Input: part model. Units: mm. Frame: model coordinates. A direction names the side the tool comes from. Round coordinates to 2 decimals unless told otherwise and drop trailing zeros. Order: outer loops, then holes, each group sorted by start corner. A loop starts at its lowest first (then second) coordinate and runs counter-clockwise, first axis right, second up. Notation, with made-up numbers: (4.5, -4.75) -> (48.5, -4.75) arc R21 cw to (48.5, 10.25) -> close; hole circle Ø1 at (23.5, 1.5). An arc over 180 degrees is marked (long way). Use a Markdown table: item, result.
from build123d import *

# Parameters (mm, degrees)
SKETCH1_R           = 35
SKETCH1_R_2         = 27.75
BOSS_EXTRUDE1_DEPTH = 6.5
CUT_EXTRUDE1_DEPTH  = 50.922439844
CHAMFER1_SIZE       = 2
CHAMFER2_SIZE       = 0.5


with BuildPart() as part:
    # Sketch1 → Boss-Extrude1 (new body)
    with BuildSketch(Plane.XY):
        with Locations(Location((0, 0, 0), (0, 0, 180))):
            Circle(SKETCH1_R)
        with Locations(Location((0, 0, 0), (0, 0, 180))):
            Circle(SKETCH1_R_2, mode=Mode.SUBTRACT)
    extrude(amount=BOSS_EXTRUDE1_DEPTH)

    # Sketch2 → Cut-Extrude1 (cut, through all)
    with BuildSketch(Plane.XY.offset(6.5)):
        Polygon((0, 0), (8.5, 0), (8.5, 53.904694855), (-8.5, 53.904694855), (-8.5, 0), align=None)
    extrude(amount=-CUT_EXTRUDE1_DEPTH, mode=Mode.SUBTRACT)

    # Chamfer1
    chamfer1_edges = [part.edges().sort_by_distance(p)[0] for p in [
        (0, -27.75, 0),
        (0, -27.75, 6.5),
    ]]
    chamfer(chamfer1_edges, length=CHAMFER1_SIZE)

    # Chamfer2
    chamfer2_edges = [part.edges().sort_by_distance(p)[0] for p in [
        (0, -35, 6.5),
        (0, -35, 0),
    ]]
    chamfer(chamfer2_edges, length=CHAMFER2_SIZE)


solid = part.part
1) Line query: L1, parallel to X at y = 0, z = 3.2; L2, parallel to X at y = -4.5, z = 3.5; L3, parallel to Y at x = -20.5, z = 0.5. Output: solid intervals per line, ascending. Write a range as [from, to].
Results found:
| item | result |
|---|---|
| L1 | x = [-35, -27.75], [27.75, 35] |
| L2 | x = [-34.71, -27.38], [27.38, 34.71] |
| L3 | y = [-28.37, -20.86], [20.86, 28.37] |
2) Pull-direction query (X, two-part tool) for faces 1 (the conical face through (-1.4, -34.61, 0.14)), 2 (the flat face through (-15, -26, 0)), 3 (the flat face through (-8.5, 30, 3)); classes: +X half, -X half, draft (parallel to the pull), parting line (faces both ways), or undercut.
Results found:
| item | result |
|---|---|
| face 1 | parting line |
| face 2 | draft |
| face 3 | undercut |
3) Set-up query: faces 4 (the flat face through (8.5, 30, 3)), 5 (the cylindrical face through (-1.1, -27.73, 3.23)). Return all of +Z, -Z, +X, -X, +Y, -Y with unobstructed straight access to the full face (end or side cutting, diameter ignored); none if empty.
Results found:
| item | result |
|---|---|
| face 4 | +Z, -Z, +Y |
| face 5 | +Z, -Z |
4) Pin query (flat end, axial travel): pin 1 Ø2 at (y, z) = (30, 3) entering from -X; pin 2 Ø3 at (x, z) = (26, 4) entering from -Y (3 decimals); pin 3 Ø3 at (y, z) = (21, 3) entering from +X. Return the tip coordinate at first contact, or that it passes through.
Results found:
| item | result |
|---|---|
| pin 1 | stops at x = -19.6 |
| pin 2 | stops at y = -24.995 |
| pin 3 | stops at x = 29.06 |
5) Cut plane A-A on y = 0. Return loops of the section in (x, z), and give its area (4 significant figures).
Results found:
| item | result |
|---|---|
| outline | (-35, 0.5) -> (-34.5, 0) -> (-29.75, 0) -> (-27.75, 2) -> (-27.75, 4.5) -> (-29.75, 6.5) -> (-34.5, 6.5) -> (-35, 6) -> close; (27.75, 2) -> (29.75, 0) -> (34.5, 0) -> (35, 0.5) -> (35, 6) -> (34.5, 6.5) -> (29.75, 6.5) -> (27.75, 4.5) -> close |
| area | 85.75 mm² |
